```python
from build123d import *

# Parameters (mm, degrees)
SKETCH_1_R          = 3.5
EXTRUDE_1_DEPTH     = 4
CUT_EXTRUDE_1_DEPTH = 2
FILLET_1_R          = 0.2
SKETCH_5_R          = 2
EXTRUDE_2_DEPTH     = 14
CHAMFER_2_SIZE      = 0.39


with BuildPart() as part:
    # 草图1 → 凸台-拉伸1 (new body)
    with BuildSketch(Plane(origin=(0, 0, 0), x_dir=(1, 0, 0), z_dir=(0, 1, 0))):
        with Locations(Location((0, 0, 0), (0, 0, 270))):
            Circle(SKETCH_1_R)
    extrude(amount=EXTRUDE_1_DEPTH)

    # 草图2 → 切除-拉伸1 (cut)
    with BuildSketch(Plane(origin=(0, 4, 0), x_dir=(1, 0, 0), z_dir=(0, 1, 0))):
        Polygon((1.772465326, 0), (0.886232663, 1.535), (-0.886232663, 1.535), (-1.772465326, 0), (-0.886232663, -1.535), (0.886232663, -1.535), align=None)
    extrude(amount=-CUT_EXTRUDE_1_DEPTH, mode=Mode.SUBTRACT)

    # 圆角1
    fillet_1_edges = [part.edges().sort_by_distance(p)[0] for p in [
        (0, 4, -3.5),
    ]]
    fillet(fillet_1_edges, radius=FILLET_1_R)

    # 草图5 → 凸台-拉伸2 (add)
    with BuildSketch(Plane.XZ):
        with Locations(Location((0, 0, 0), (0, 0, 90))):
            Circle(SKETCH_5_R)
    extrude(amount=EXTRUDE_2_DEPTH)

    # 倒角2
    chamfer_2_edges = [part.edges().sort_by_distance(p)[0] for p in [
        (0, -14, -2),
    ]]
    chamfer(chamfer_2_edges, length=CHAMFER_2_SIZE)


solid = part.part
```
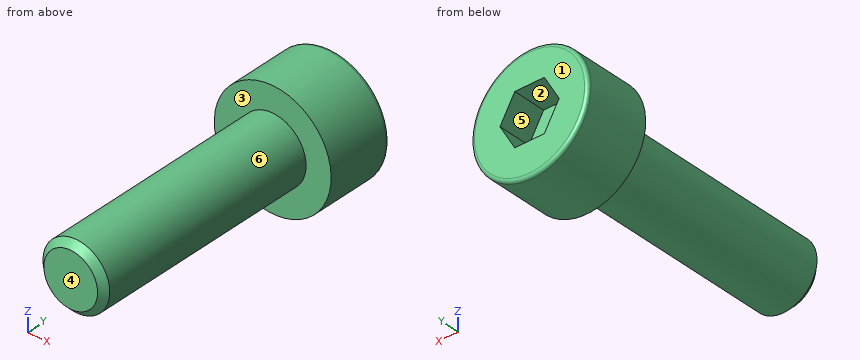
Geometry check sheet. Reference: the model listing, model coordinates, mm. Face numbers are marked on the shaded views. A direction names the side the tool comes from. Round coordinates to 2 decimals unless told otherwise and drop trailing zeros. Loops run counter-clockwise (first coordinate to the right, second up) from the corner with the lowest first, then second, coordinate; pieces in that order, holes last. Notation, with made-up numbers: (-24.5, 61) - (14.5, 61) arc R28 ccw to (14.5, 97) - close; hole circle Ø9 at (57, -25.75). An arc over 180 degrees is marked (long way). Use a Markdown table: item, result.
Q1. Access from +Z, -Z, +X, -X, +Y, -Y to the whole of each face (thin tool, end or side, straight path). Record for the marked faces 1, 2 and 3.
Solutions:
| item | result |
|---|---|
| face 1 | +Z, -Z, +X, -X, +Y |
| face 2 | +Y |
| face 3 | -Y |
Q2. Material ranges on line 1 (Y direction, x = 1, z = -1.25); line 2 (Y direction, x = -2, z = -2.5); line 3 (Z direction, x = -0.25, y = 2.75) (3 decimals), recorded low to high.
Solutions:
| item | result |
|---|---|
| line 1 | y = -14 to 2 |
| line 2 | y = 0 to 4 |
| line 3 | z = -3.491 to -1.535, 1.535 to 3.491 |
Q3. Cross-section at B-B on y = -5.25. Record the cut outline in (x, z).
Solutions:
| item | result |
|---|---|
| outline | circle Ø4 at (0, 0) |
Q4. Draft check along X on the marked faces 4, 5 and 6. Enter one of: released by +X, released by -X, zero draft, split by the parting line, or undercut.
Solutions:
| item | result |
|---|---|
| face 4 | zero draft |
| face 5 | undercut |
| face 6 | split by the parting line |
Q5. Go/stop test with flat-tipped pins: P1, Ø0.5, axis at x = 0.5, y = 3, coming from the -Z side; P2, Ø1, axis at x = 0, y = -2.5, coming from the -Z side; P3, Ø0.9, axis at x = 0.5, z = 0.5, coming from the +Y side. Record where each tip stops, or that it passes through.
Solutions:
| item | result |
|---|---|
| P1 | stops at z = -3.49 |
| P2 | stops at z = -2 |
| P3 | stops at y = 2 |
Q6. Cross-section at A-A on x = 0. Record the cut outline in (y, z) (3 decimals), plus the area to 3 significant figures.
Solutions:
| item | result |
|---|---|
| outline | (-14, -1.61) - (-13.61, -2) - (0, -2) - (0, -3.5) - (3.8, -3.5) arc R0.2 ccw to (4, -3.3) - (4, -1.535) - (2, -1.535) - (2, 1.535) - (4, 1.535) - (4, 3.3) arc R0.2 ccw to (3.8, 3.5) - (0, 3.5) - (0, 2) - (-13.61, 2) - (-14, 1.61) - close |
| area | 77.7 mm2 |
Q7. Cross-section at C-C on y = 0.5. Record the cut outline in (x, z).
Solutions:
| item | result |
|---|---|
| outline | circle Ø7 at (0, 0) |
